Geometry check sheet. Reference: the model listing, model coordinates, mm. Face numbers are marked on the shaded views. Give positions to 0.01 mm unless a question says otherwise; leave off trailing zeros. Write each loop counter-clockwise with the first axis right and the second up, starting at its lowest first coordinate (ties: lowest second). Pieces come first, ordered by that corner, then holes. Notation, with made-up numbers: (9.25, -24.5) - (21.25, -24.5) arc R23 ccw to (21.25, 11.5) - close; hole circle Ø7 at (-18.75, 29.5). An arc over 180 degrees is marked (long way). One line per question, with ' | ' between items. Start each with the question number.
Q1. Thickness scan on L1, parallel to X at y = 7.5, z = 334; L2, parallel to Y at x = -56, z = 491; L3, parallel to X at y = 4.75, z = 414. Record the ranges inside material, lowest first. Write a range as [from, to].
Q2. Section check A-A on y = 2. Record the boundary of the cut face in (x, z), and give its area (3 significant figures).
Q3. Section check B-B on z = 415. Record the boundary of the cut face in (x, y), and give its area (3 significant figures).
Q4. Release check for a two-part mould opening along X. For the marked faces 1 and 2 record: +X half, -X half, draft (parallel to the pull), parting line (faces both ways), or undercut.
Q5. Section check C-C on x = -4. Record the boundary of the cut face in (y, z).
Q6. Gauge pin test, flat ends, axial feed: P1, Ø5, axis at x = 32.5, y = 5, coming from the -Z side; P2, Ø1.5, axis at x = -3, z = -348.5, coming from the -Y side; P3, Ø1.5, axis at x = -56, z = 38, coming from the -Y side; P4, Ø1.2, axis at x = 54, z = -192, coming from the -Y side. Record the tip position at first contact, or that the pin passes through.
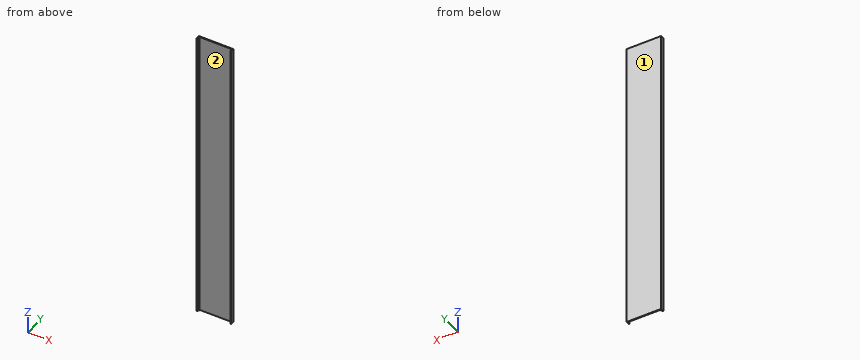
```python
from build123d import *

# Parameters (mm, degrees)
SKETCH_1_R                  = 1.25
EXTRUDE_1_DEPTH             = 500
CUT_EXTRUDE_1_DEPTH         = 504.730086455
CUT_EXTRUDE_1_DEPTH_BACK    = 504.730086455
SKETCH_2_W                  = 1.7
SKETCH_2_H                  = 1.9
HOLE_WIZARD_M3_1_AT_2_COUNT = 2
HOLE_WIZARD_M3_1_AT_2_PITCH = 112


with BuildPart() as part:
    # 草图1 → 凸台-拉伸1 (new, symmetric)
    with BuildSketch(Plane.XY):
        Polygon((60, 12), (-60, 12), (-60, 0), (-56.8, 0), (-56.8, 5.5), (-53.7, 5.5), (-53.7, 9), (53.7, 9), (53.7, 5.5), (56.8, 5.5), (56.8, 0), (60, 0), align=None)
        with Locations((-56, 7.7)):
            Circle(SKETCH_1_R, mode=Mode.SUBTRACT)
        with Locations(Location((56, 7.7, 0), (0, 0, 180))):
            Circle(SKETCH_1_R, mode=Mode.SUBTRACT)
    extrude(amount=EXTRUDE_1_DEPTH, both=True)

    # 草图2 → 切除-拉伸1 (cut, two sides: drawn at the far end of the back side and taken through both)
    with BuildSketch(Plane.XY.offset(-CUT_EXTRUDE_1_DEPTH_BACK)):
        with Locations((-54.55, 6.45)):
            Rectangle(SKETCH_2_W, SKETCH_2_H)
        with Locations((54.55, 6.45)):
            Rectangle(SKETCH_2_W, SKETCH_2_H)
    extrude(amount=CUT_EXTRUDE_1_DEPTH + CUT_EXTRUDE_1_DEPTH_BACK, mode=Mode.SUBTRACT)

    # 草图7 → M3 螺纹孔1 (revolve, cut)
    with BuildSketch(Plane(origin=(-56, 7.7, 500), x_dir=(0, -1, 0), z_dir=(1, 0, 0))):
        Polygon((0, 0), (0, 20.781118805), (1.3, 20), (1.3, 0), align=None)
    hole_wizard_m3_1 = revolve(axis=Axis((-56, 7.7, 506.35), (0, 0, -1)), mode=Mode.SUBTRACT)

    # M3 螺纹孔1 at 2: M3 螺纹孔1 ×2
    with Locations(*[(i * HOLE_WIZARD_M3_1_AT_2_PITCH, 0, 0) for i in range(1, HOLE_WIZARD_M3_1_AT_2_COUNT)]):
        add(hole_wizard_m3_1, mode=Mode.SUBTRACT)

    # 镜向1: M3 螺纹孔1 across plane
    add(hole_wizard_m3_1.mirror(Plane.XY), mode=Mode.SUBTRACT)

    # 镜向1 copy 1 sketch → 镜向1 copy 1 (revolve, cut)
    with BuildSketch(Plane(origin=(56, 7.7, -500), x_dir=(0, -1, 0), z_dir=(1, 0, 0))):
        Polygon((0, 0), (0, -20.781118805), (1.3, -20), (1.3, 0), align=None)
    revolve(axis=Axis((56, 7.7, -506.35), (0, 0, -1)), mode=Mode.SUBTRACT)


solid = part.part
```
Working result:
1) L1: x = [-60, -57.23], [-54.77, -53.7], [53.7, 54.77], [57.23, 60] | L2: y = [5.5, 6.4], [9, 12] | L3: x = [-60, -56.8], [56.8, 60]
2) outline: (-60, -500) - (-56.8, -500) - (-56.8, 500) - (-60, 500) - close; (56.8, -500) - (60, -500) - (60, 500) - (56.8, 500) - close | area: 6,400 mm2
3) outline: (-60, 0) - (-56.8, 0) - (-56.8, 5.5) - (-55.4, 5.5) - (-55.4, 6.6) arc R1.25 cw (long way) to (-54.79, 7.4) - (-53.7, 7.4) - (-53.7, 9) - (53.7, 9) - (53.7, 7.4) - (54.79, 7.4) arc R1.25 cw (long way) to (55.4, 6.6) - (55.4, 5.5) - (56.8, 5.5) - (56.8, 0) - (60, 0) - (60, 12) - (-60, 12) - close | area: 424 mm2
4) face 1: draft | face 2: undercut
5) outline: (9, -500) - (12, -500) - (12, 500) - (9, 500) - close
6) P1: passes through | P2: stops at y = 9 | P3: stops at y = 5.5 | P4: stops at y = 7.4
